Part model, mm, in its own coordinate system. A direction names the side the tool comes from. Round coordinates to 2 decimals unless told otherwise and drop trailing zeros. Loops run counter-clockwise (first coordinate to the right, second up) from the corner with the lowest first, then second, coordinate; pieces in that order, holes last. Notation, with made-up numbers: M 63.5,51 L 79.5,51 A22 cw 79.5,90 Z; hole C -26,79 d3. An arc over 180 degrees is marked long. Put each result on its own line as item: value. Start each with the question number.
```python
from build123d import *

# Parameters (mm, degrees)
SKETCH1_R                             = 80
BOSS_EXTRUDE1_DEPTH                   = 75
SKETCH2_OUTSIDE_W                     = 209.676
SKETCH2_OUTSIDE_H                     = 209.676
SKETCH2_OUTSIDE_W_2                   = 199.64377861
SKETCH2_OUTSIDE_H_2                   = 130
CUT_EXTRUDE1_DEPTH                    = 136.738719605
CUT_EXTRUDE2_DEPTH                    = 131.096118313
CUT_EXTRUDE3_DEPTH                    = 8
CUT_EXTRUDE4_START                    = -59
CUT_EXTRUDE4_DEPTH                    = 8
M6_TAPPED_HOLE1_D                     = 5
M6_TAPPED_HOLE1_DEPTH                 = 15
M6_TAPPED_HOLE1_CSINK_D               = 6.05
M6_TAPPED_HOLE1_CSINK_ANGLE           = 90
M6_TAPPED_HOLE1_TIP                   = 1.502151548
M6_TAPPED_HOLE1_ON_FACE_2_D           = 5
M6_TAPPED_HOLE1_ON_FACE_2_DEPTH       = 15
M6_TAPPED_HOLE1_ON_FACE_2_CSINK_D     = 6.05
M6_TAPPED_HOLE1_ON_FACE_2_CSINK_ANGLE = 90
M6_TAPPED_HOLE1_ON_FACE_2_TIP         = 1.502151548
CUT_EXTRUDE5_REACH                    = 172.074
SKETCH7_R                             = 12.1
BOSS_EXTRUDE4_START                   = 8
SKETCH8_R                             = 25
SKETCH8_R_2                           = 12.1
BOSS_EXTRUDE4_DEPTH                   = 8


with BuildPart() as part:
    # Sketch1 → Boss-Extrude1 (new body)
    with BuildSketch(Plane.XY):
        Circle(SKETCH1_R)
    extrude(amount=BOSS_EXTRUDE1_DEPTH)

    # Sketch2 outside → Cut-Extrude1 (cut, through all)
    with BuildSketch(Plane(origin=(0, 0, 0), x_dir=(-1, 0, 0), z_dir=(0, 0, -1))):
        Rectangle(SKETCH2_OUTSIDE_W, SKETCH2_OUTSIDE_H)
        with Locations((0.958801498, -5)):
            Rectangle(SKETCH2_OUTSIDE_W_2, SKETCH2_OUTSIDE_H_2, mode=Mode.SUBTRACT)
    extrude(amount=-CUT_EXTRUDE1_DEPTH, mode=Mode.SUBTRACT)

    # Sketch3 → Cut-Extrude2 (cut, through all)
    with BuildSketch(Plane(origin=(0, 0, 0), x_dir=(-1, 0, 0), z_dir=(0, 0, -1))):
        with BuildLine():
            Line((-25, -70), (-45, 5))
            ThreePointArc((-45, 5), (-52.5, 12.5), (-45, 20))
            Line((-45, 20), (45, 20))
            ThreePointArc((45, 20), (52.5, 12.5), (45, 5))
            Line((45, 5), (25, -70))
            Line((25, -70), (-25, -70))
        make_face()
    extrude(amount=-CUT_EXTRUDE2_DEPTH, mode=Mode.SUBTRACT)

    # Sketch4 → Cut-Extrude3 (cut)
    with BuildSketch(Plane(origin=(0, 0, 0), x_dir=(-1, 0, 0), z_dir=(0, 0, -1))):
        with BuildLine():
            Line((-45, -23), (45, -23))
            ThreePointArc((45, -23), (53, -31), (45, -39))
            Line((45, -39), (-45, -39))
            ThreePointArc((-45, -39), (-53, -31), (-45, -23))
        make_face()
    extrude(amount=-CUT_EXTRUDE3_DEPTH, mode=Mode.SUBTRACT)

    # Sketch5 → Cut-Extrude4 (cut)
    with BuildSketch(Plane(origin=(0, 0, 8), x_dir=(-1, 0, 0), z_dir=(0, 0, -1)).offset(CUT_EXTRUDE4_START)):
        with BuildLine():
            Line((37.533333333, -23), (33.266666667, -39))
            Line((33.266666667, -39), (45, -39))
            ThreePointArc((45, -39), (53, -31), (45, -23))
            Line((45, -23), (37.533333333, -23))
        make_face()
        with BuildLine():
            Line((-33.266666667, -39), (-37.533333333, -23))
            Line((-37.533333333, -23), (-45, -23))
            ThreePointArc((-45, -23), (-53, -31), (-45, -39))
            Line((-45, -39), (-33.266666667, -39))
        make_face()
    extrude(amount=-CUT_EXTRUDE4_DEPTH, mode=Mode.SUBTRACT)

    # M6 Tapped Hole1
    with Locations(Plane(origin=(45, -31, 8), x_dir=(-1, 0, 0), z_dir=(0, 0, -1))):
        with Locations((0, 0), (90, 0)):
            CounterSinkHole(M6_TAPPED_HOLE1_D / 2, M6_TAPPED_HOLE1_CSINK_D / 2, depth=M6_TAPPED_HOLE1_DEPTH, counter_sink_angle=M6_TAPPED_HOLE1_CSINK_ANGLE)
            with Locations((0, 0, -(M6_TAPPED_HOLE1_DEPTH + M6_TAPPED_HOLE1_TIP / 2))):  # 118° drill point
                Cone(0, M6_TAPPED_HOLE1_D / 2, M6_TAPPED_HOLE1_TIP, mode=Mode.SUBTRACT)

    # M6 Tapped Hole1 on face 2
    with Locations(Plane(origin=(-45, -31, 67), x_dir=(1, 0, 0), z_dir=(0, 0, 1))):
        with Locations((0, 0), (90, 0)):
            CounterSinkHole(M6_TAPPED_HOLE1_ON_FACE_2_D / 2, M6_TAPPED_HOLE1_ON_FACE_2_CSINK_D / 2, depth=M6_TAPPED_HOLE1_ON_FACE_2_DEPTH, counter_sink_angle=M6_TAPPED_HOLE1_ON_FACE_2_CSINK_ANGLE)
            with Locations((0, 0, -(M6_TAPPED_HOLE1_ON_FACE_2_DEPTH + M6_TAPPED_HOLE1_ON_FACE_2_TIP / 2))):  # 118° drill point
                Cone(0, M6_TAPPED_HOLE1_ON_FACE_2_D / 2, M6_TAPPED_HOLE1_ON_FACE_2_TIP, mode=Mode.SUBTRACT)

    # Sketch7 → Cut-Extrude5 (cut, up to next)
    with BuildSketch(Plane(origin=(0, 60, 0), x_dir=(1, 0, 0), z_dir=(0, 1, 0)), mode=Mode.PRIVATE) as cut_extrude5_sk1:
        with Locations(Location((0, -37.5, 0), (0, 0, 270))):
            Circle(SKETCH7_R)
    cut_extrude5_tool1 = extrude(cut_extrude5_sk1.sketch, amount=-CUT_EXTRUDE5_REACH, mode=Mode.PRIVATE) & part.part
    add(cut_extrude5_tool1.solids().sort_by_distance((0, 60, 37.5))[0], mode=Mode.SUBTRACT)

    # Sketch8 → Boss-Extrude4 (add)
    with BuildSketch(Plane(origin=(0, 60, 0), x_dir=(1, 0, 0), z_dir=(0, 1, 0)).offset(BOSS_EXTRUDE4_START)):
        with Locations(Location((0, -37.5, 0), (0, 0, 270))):
            Circle(SKETCH8_R)
        with Locations(Location((0, -37.5, 0), (0, 0, 270))):
            Circle(SKETCH8_R_2, mode=Mode.SUBTRACT)
    extrude(amount=-BOSS_EXTRUDE4_DEPTH)


solid = part.part
```
1. Mould opens along X. For faces 5 (the flat face through (-39, -39, 71)), 6 (the cylindrical face through (79.405, -9.742, 36.975)), 7 (the flat face through (24, 60, 29)) say: released by +X, released by -X, zero draft, split by the parting line, or undercut.
2. Wall check: L1, parallel to Y at x = 50.5, z = 7; L2, parallel to Y at x = 45.5, z = 10; L3, parallel to X at y = -11, z = 50.5. Give the ranges that are in metal, low to high.
3. Which spindle directions (+Z, -Z, +X, -X, +Y, -Y) get a long thin tool onto all of the face, cutting with end or side? Do faces 1 (the flat face through (-1, 25, 75)), 2 (the cylindrical face through (-52.5, 12.66, 36.98)), 3 (the flat face through (39, -39, 4)), 4 (the flat face through (-41, -23, 71)). Say none if no direction does.
4. Cut at A-A, the plane x = 0. Give the cut face in (y, z).
5. Cut at C-C, the plane y = -18. Give the cut face in (x, z), and give its area (3 significant figures).
6. Cut at D-D, the plane z = 15. Give the cut face in (x, y), and give its area (3 significant figures).
7. Cut at B-B, the plane z = 37.5. Give the cut face in (x, y), and give its area (3 significant figures).
8. Drop flat-ended pins along their axis: pin 1 (2 mm diameter, centred on y = -47, z = 38.5, fed in from -X); pin 2 (8 mm diameter, centred on x = -46, y = -28.5, fed in from +Z); pin 3 (2 mm diameter, centred on x = -41.5, z = 2.5, fed in from -Y). Give the stop position or say it passes through.
Results list:
1. face 5: undercut
1. face 6: released by +X
1. face 7: zero draft
2. L1: y = -62.05 to -36.81, -25.19 to 7.4, 17.6 to 60
2. L2: y = -65.8 to -33.45, -28.55 to 5.02, 19.98 to 60
2. L3: x = -79.24 to -40.73, 40.73 to 79.24
3. face 1: +Z, +X, -X, +Y, -Y
3. face 2: +Z, -Z
3. face 3: -Z
3. face 4: +Z
4. outline: M 20,0 L 60,0 L 60,12.5 L 68,12.5 L 68,25.4 L 20,25.4 Z; M 20,49.6 L 68,49.6 L 68,62.5 L 60,62.5 L 60,75 L 20,75 Z
5. outline: M -77.95,0 L -38.87,0 L -38.87,75 L -77.95,75 Z; M 38.87,0 L 77.95,0 L 77.95,75 L 38.87,75 Z
5. area: 5,860 mm^2
6. outline: M -52.92,60 A80 ccw -38.73,-70 L -25,-70 L -45,5 A7.5 cw -45,20 L 45,20 A7.5 cw 45,5 L 25,-70 L 38.73,-70 A80 ccw 52.92,60 L 10.9,60 L 10.9,68 L -10.9,68 L -10.9,60 Z; hole C -45,-31 d5; hole C 45,-31 d5
6. area: 11,500 mm^2
7. outline: M -52.92,60 A80 ccw -38.73,-70 L -25,-70 L -45,5 A7.5 cw -45,20 L -12.1,20 L -12.1,68 L -25,68 L -25,60 Z; M 12.1,20 L 45,20 A7.5 cw 45,5 L 25,-70 L 38.73,-70 A80 ccw 52.92,60 L 25,60 L 25,68 L 12.1,68 Z
7. area: 10,600 mm^2
8. pin 1: stops at x = -65.45
8. pin 2: stops at z = 67
8. pin 3: stops at y = -68.99
